Design review of the part shown in the three views and the two pictorial views. Dimensions are in mm from the part's minimum x, y and z. A direction names the side the tool comes from. Round coordinates to 2 decimals unless told otherwise and drop trailing zeros. Write each loop counter-clockwise with the first axis right and the second up, starting at its lowest first coordinate (ties: lowest second). Pieces come first, ordered by that corner, then holes. Notation, with made-up numbers: (-25.75, 1.25) - (27.25, 1.25) arc R28 ccw to (27.25, 22.25) - close; hole circle Ø8 at (53.5, 33.5). An arc over 180 degrees is marked (long way). One line per item, written item: value. Start each with the question number.
Q1. Add section C-C on z = 22.75. Write out the cut boundary in (x, y).
Q2. Tool access review of the marked faces 1, 2 and 3: name each direction out of +Z, -Z, +X, -X, +Y, -Y from which nothing blocks a thin tool from reaching the whole face with its end or side.
Q3. Add section A-A on y = 12.5. Write out the cut boundary in (x, z), and give its area (3 significant figures).
Q4. Clearance check with flat-ended pins moving along their axes: pin 1 Ø1 at (x, z) = (23, 15) entering from -Y; pin 2 Ø10 at (y, z) = (30, 20.5) entering from +X; pin 3 Ø8 at (x, y) = (152.5, 25) entering from +Z; pin 4 Ø5 at (x, y) = (179, 25) entering from -Z. State where each tip first meets the part, or that it passes through.
Q5. Add section D-D on x = 152.5. Write out the cut boundary in (y, z), and give its area (3 significant figures).
Q6. Add section B-B on x = 115. Write out the cut boundary in (y, z).
Q7. For probe 1 along Y at (x, z) = (115, 4.35); probe 2 along Y at (x, z) = (70, 21); probe 3 along Y at (x, z) = (152.5, 11.5), list the stretches that pass through material, from the lowest coordinate up.
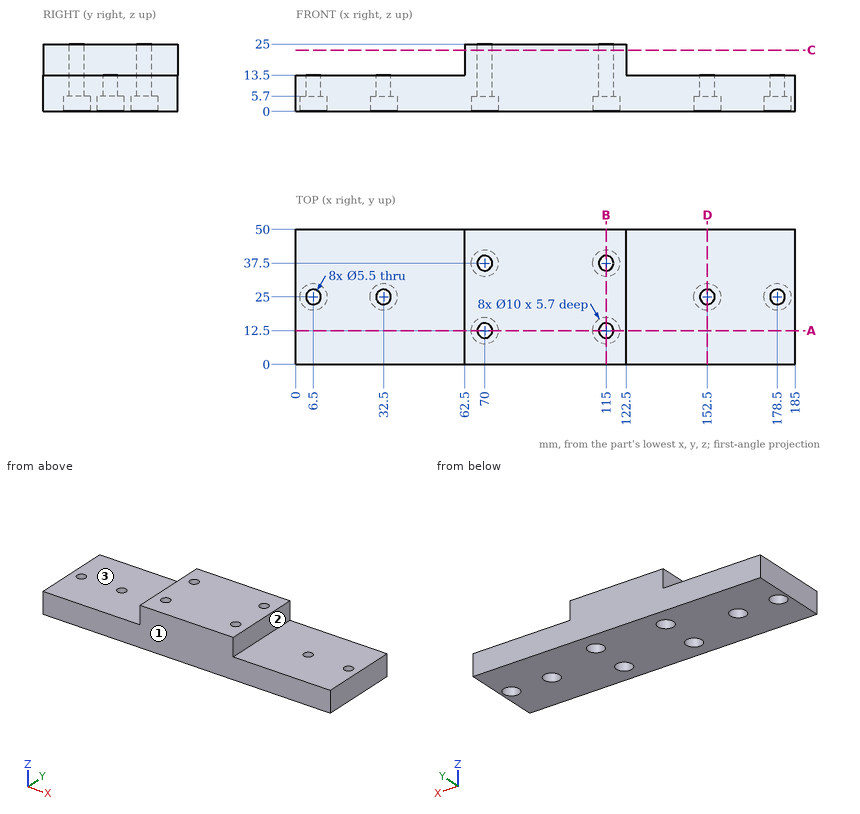
Result set:
1. outline: (62.5, 0) - (122.5, 0) - (122.5, 50) - (62.5, 50) - close; hole circle Ø5.5 at (70, 12.5); hole circle Ø5.5 at (70, 37.5); hole circle Ø5.5 at (115, 12.5); hole circle Ø5.5 at (115, 37.5)
2. face 1: +Z, -Z, +X, -X, -Y
2. face 2: +Z, +X, +Y, -Y
2. face 3: +Z, -X, +Y, -Y
3. outline: (0, 0) - (65, 0) - (65, 5.7) - (67.25, 5.7) - (67.25, 25) - (62.5, 25) - (62.5, 13.5) - (0, 13.5) - close; (72.75, 5.7) - (75, 5.7) - (75, 0) - (110, 0) - (110, 5.7) - (112.25, 5.7) - (112.25, 25) - (72.75, 25) - close; (117.75, 5.7) - (120, 5.7) - (120, 0) - (185, 0) - (185, 13.5) - (122.5, 13.5) - (122.5, 25) - (117.75, 25) - close
3. area: 2,860 mm^2
4. pin 1: passes through
4. pin 2: stops at x = 122.5
4. pin 3: stops at z = 13.5
4. pin 4: stops at z = 5.7
5. outline: (0, 0) - (20, 0) - (20, 5.7) - (22.25, 5.7) - (22.25, 13.5) - (0, 13.5) - close; (27.75, 5.7) - (30, 5.7) - (30, 0) - (50, 0) - (50, 13.5) - (27.75, 13.5) - close
5. area: 575 mm^2
6. outline: (0, 0) - (7.5, 0) - (7.5, 5.7) - (9.75, 5.7) - (9.75, 25) - (0, 25) - close; (15.25, 5.7) - (17.5, 5.7) - (17.5, 0) - (32.5, 0) - (32.5, 5.7) - (34.75, 5.7) - (34.75, 25) - (15.25, 25) - close; (40.25, 5.7) - (42.5, 5.7) - (42.5, 0) - (50, 0) - (50, 25) - (40.25, 25) - close
7. probe 1: y = 0 to 7.5, 17.5 to 32.5, 42.5 to 50
7. probe 2: y = 0 to 9.75, 15.25 to 34.75, 40.25 to 50
7. probe 3: y = 0 to 22.25, 27.75 to 50
